Design review of the part built by this model. Coordinates are the model's own, in mm. A direction names the side the tool comes from. Give positions to 0.01 mm unless a question says otherwise; leave off trailing zeros. Use a Markdown table: item, result. Add a question column.
1. To check wall thickness, follow line 1 (Y direction, x = -275.5, z = 452); line 2 (Z direction, x = -234.5, y = 956.5); line 3 (Z direction, x = -299.5, y = 953.5). State the ranges of each line that lie inside material, in increasing order.
2. For pin 1 Ø1.2 at (x, z) = (-140, 451.5) entering from +Y; pin 2 Ø0.8 at (x, z) = (-213, 457) entering from +Y; pin 3 Ø8 at (x, y) = (-122.5, 959.5) entering from +Z, all flat-tipped, find the tip position at first contact; note any pin that passes through.
3. For faces 1 (the flat face through (31.5, 960.6, 455.6)), 2 (the flat face through (-199, 961, 456)), list the 3-axis set-ups (+Z, -Z, +X, -X, +Y, -Y) from which the entire face can be reached by the end or side of a thin tool; tool diameter is ignored.
4. Draft analysis for pull direction Z (two halves, no side actions). For faces 3 (the flat face through (-199, 963, 455.2)), 4 (the flat face through (-199, 959, 451.1)), 5 (the flat face through (-423.5, 960.6, 455.6)), state which applies: pulls with the +Z half, pulls with the -Z half, needs draft (parallel to the pull), parting line crosses it, or undercut.
```python
from build123d import *

# Parameters (mm, degrees)
BOSS_EXTRUDE1_DEPTH = 455


with BuildPart() as part:
    # Sketch1 → Boss-Extrude1 (new body)
    with BuildSketch(Plane(origin=(-423.5, 0, 0), x_dir=(0, -1, 0), z_dir=(-1, 0, 0))):
        with BuildLine():
            Line((-955, 454.95), (-955, 452.15))
            ThreePointArc((-955, 452.15), (-955.073223305, 451.973223305), (-955.25, 451.9))
            Line((-955.25, 451.9), (-961.9, 451.9))
            Line((-961.9, 451.9), (-961.9, 452.7))
            Line((-961.9, 452.7), (-962.45, 452.7))
            ThreePointArc((-962.45, 452.7), (-962.626776695, 452.626776695), (-962.7, 452.45))
            Line((-962.7, 452.45), (-962.7, 451.35))
            ThreePointArc((-962.7, 451.35), (-962.626776695, 451.173223305), (-962.45, 451.1))
            Line((-962.45, 451.1), (-955.2, 451.1))
            ThreePointArc((-955.2, 451.1), (-954.492893219, 451.392893219), (-954.2, 452.1))
            Line((-954.2, 452.1), (-954.2, 453.373491886))
            ThreePointArc((-954.2, 453.373491886), (-953.665028159, 454.665028159), (-952.373491886, 455.2))
            Line((-952.373491886, 455.2), (-952.3, 455.2))
            ThreePointArc((-952.3, 455.2), (-951.592893219, 455.492893219), (-951.3, 456.2))
            Line((-951.3, 456.2), (-951.3, 458.6))
            ThreePointArc((-951.3, 458.6), (-951.739339828, 459.660660172), (-952.8, 460.1))
            Line((-952.8, 460.1), (-953.2, 460.1))
            ThreePointArc((-953.2, 460.1), (-954.191183271, 459.232498012), (-953.462659626, 458.135111446))
            Line((-953.462659626, 458.135111446), (-952.837340374, 457.964888554))
            ThreePointArc((-952.837340374, 457.964888554), (-952.108816729, 456.867501988), (-953.1, 456))
            Line((-953.1, 456), (-968.799810447, 456))
            ThreePointArc((-968.799810447, 456), (-969.790988627, 456.867463908), (-969.062544211, 457.964868369))
            Line((-969.062544211, 457.964868369), (-968.437266236, 458.135131631))
            ThreePointArc((-968.437266236, 458.135131631), (-967.70882182, 459.232536092), (-968.7, 460.1))
            Line((-968.7, 460.1), (-969.1, 460.1))
            ThreePointArc((-969.1, 460.1), (-970.160660172, 459.660660172), (-970.6, 458.6))
            Line((-970.6, 458.6), (-970.6, 456))
            ThreePointArc((-970.6, 456), (-970.849658895, 455.534896264), (-971.243431907, 455.183337075))
            ThreePointArc((-971.243431907, 455.183337075), (-971.28533621, 455.130932577), (-971.284682745, 455.06383731))
            ThreePointArc((-971.284682745, 455.06383731), (-971.207838721, 454.956126495), (-971.086783129, 454.902720811))
            ThreePointArc((-971.086783129, 454.902720811), (-971.055207963, 454.903064362), (-971.025314114, 454.913236231))
            ThreePointArc((-971.025314114, 454.913236231), (-970.431156786, 455.135665686), (-969.8, 455.2))
            Line((-969.8, 455.2), (-955.25, 455.2))
            ThreePointArc((-955.25, 455.2), (-955.073223305, 455.126776695), (-955, 454.95))
        make_face()
    extrude(amount=-BOSS_EXTRUDE1_DEPTH)


solid = part.part
```
Taken from the geometry:
| question | item | result |
|---|---|---|
| 1 | line 1 | y = 954.21 to 955.05, 961.9 to 962.7 |
| 1 | line 2 | z = 451.1 to 451.9, 455.2 to 456 |
| 1 | line 3 | z = 454.81 to 456, 458.15 to 460.05 |
| 2 | pin 1 | stops at y = 962.7 |
| 2 | pin 2 | stops at y = 970.6 |
| 2 | pin 3 | stops at z = 456 |
| 3 | face 1 | +Z, -Z, +X, +Y, -Y |
| 3 | face 2 | +X, -X |
| 4 | face 3 | undercut |
| 4 | face 4 | pulls with the -Z half |
| 4 | face 5 | needs draft |
